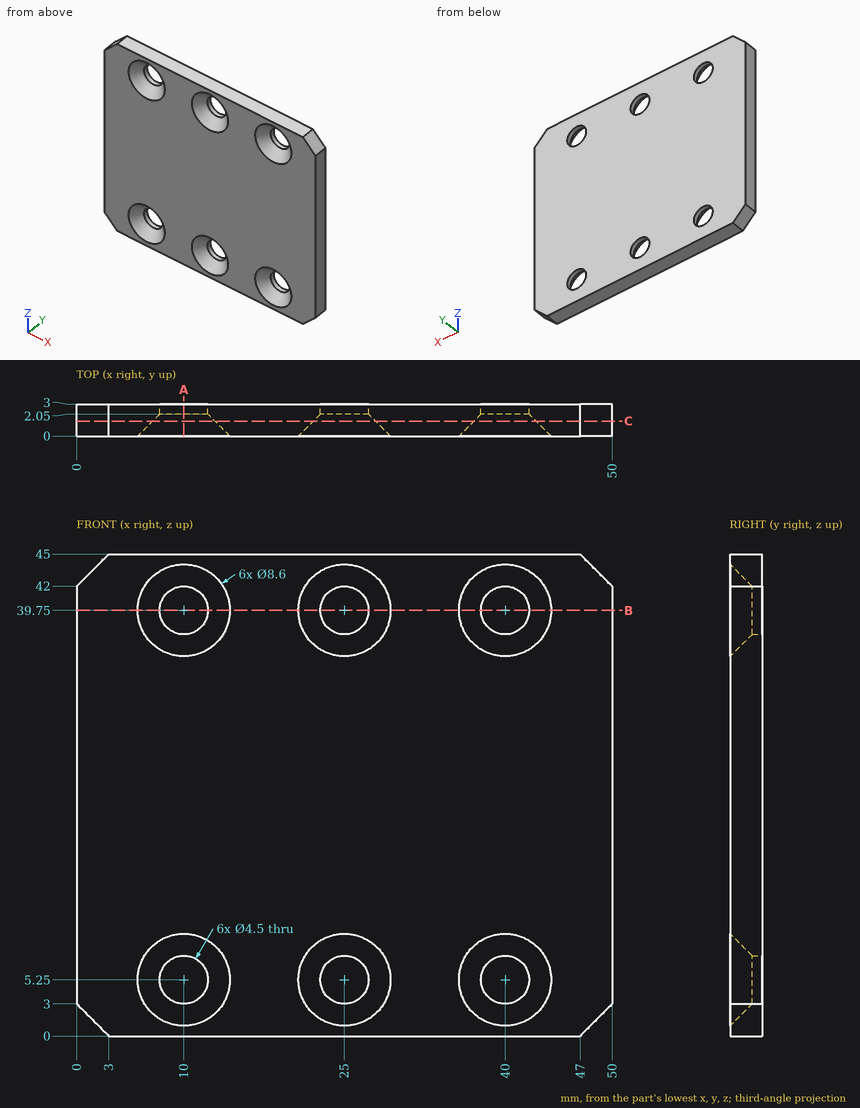
For this review, use the dimensioned drawing (mm, ordinates from the lowest corner) and the shaded views. Give positions to 0.01 mm unless a question says otherwise; leave off trailing zeros. Order: outer loops, then holes, each group sorted by start corner. A loop starts at its lowest first (then second) coordinate and runs counter-clockwise, first axis right, second up. Notation, with made-up numbers: (-26.5, 84) - (-12.5, 84) arc R32 cw to (-12.5, 115) - close; hole circle Ø6 at (52.5, 12.25). An arc over 180 degrees is marked (long way). Use CSV: the item, a comma, the result in double quotes. Start each with the question number.
Q1. We need section C-C, the plane y = 1.4. Write out the cut boundary in (x, z).
Q2. We need section B-B, the plane z = 39.75. Write out the cut boundary in (x, y).
Q3. To check wall thickness, follow line 1 along Z through (x, y) = (25, 2.3); line 2 along X through (y, z) = (2.3, 39.75); line 3 along Z through (x, y) = (23, 0.3). State the ranges of each line that lie inside material, in increasing order. Write a range as [from, to].
Q4. We need section A-A, the plane x = 10. Write out the cut boundary in (y, z), and give its area (3 significant figures).
Outcome:
1,outline,"(0, 3) - (3, 0) - (47, 0) - (50, 3) - (50, 42) - (47, 45) - (3, 45) - (0, 42) - close; hole circle Ø5.8 at (10, 5.25); hole circle Ø5.8 at (10, 39.75); hole circle Ø5.8 at (25, 5.25); hole circle Ø5.8 at (25, 39.75); hole circle Ø5.8 at (40, 5.25); hole circle Ø5.8 at (40, 39.75)"
2,outline,"(0, 0) - (5.7, 0) - (7.75, 2.05) - (7.75, 3) - (0, 3) - close; (12.25, 2.05) - (14.3, 0) - (20.7, 0) - (22.75, 2.05) - (22.75, 3) - (12.25, 3) - close; (27.25, 2.05) - (29.3, 0) - (35.7, 0) - (37.75, 2.05) - (37.75, 3) - (27.25, 3) - close; (42.25, 2.05) - (44.3, 0) - (50, 0) - (50, 3) - (42.25, 3) - close"
3,line 1,"z = [0, 3], [7.5, 37.5], [42, 45]"
3,line 2,"x = [0, 7.75], [12.25, 22.75], [27.25, 37.75], [42.25, 50]"
3,line 3,"z = [0, 1.79], [8.71, 36.29], [43.21, 45]"
4,outline,"(0, 0) - (3, 0) - (3, 3) - (2.05, 3) - (0, 0.95) - close; (0, 9.55) - (2.05, 7.5) - (3, 7.5) - (3, 37.5) - (2.05, 37.5) - (0, 35.45) - close; (0, 44.05) - (2.05, 42) - (3, 42) - (3, 45) - (0, 45) - close"
4,area,"99.6 mm^2"
